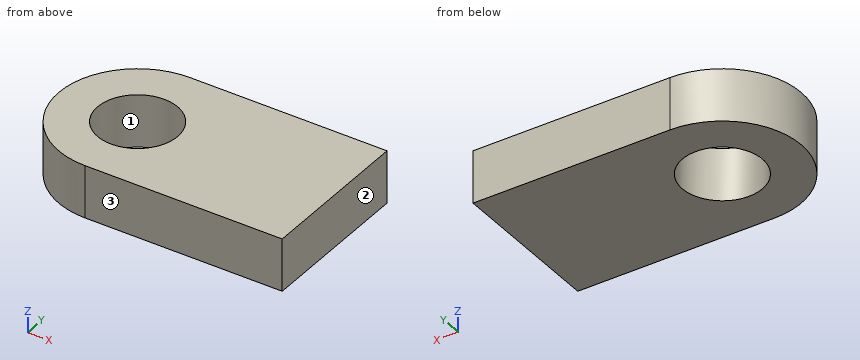
```python
from build123d import *

# Parameters (mm, degrees)
SKETCH_1_R      = 6.1
EXTRUDE_1_DEPTH = 4


with BuildPart() as part:
    # 草图1 → 凸台-拉伸1 (new, symmetric)
    with BuildSketch(Plane.XY):
        with BuildLine():
            Line((0, 12), (30, 12))
            Line((30, 12), (30, -12))
            Line((30, -12), (0, -12))
            ThreePointArc((0, -12), (-12, 0), (0, 12))
        make_face()
        Circle(SKETCH_1_R, mode=Mode.SUBTRACT)
    extrude(amount=EXTRUDE_1_DEPTH, both=True)


solid = part.part
```
Here's how the part is built. I have some questions about the finished solid (model axes, mm). Face numbers are marked on the shaded views. Give positions to 0.01 mm unless a question says otherwise; leave off trailing zeros. Write each loop counter-clockwise with the first axis right and the second up, starting at its lowest first coordinate (ties: lowest second). Pieces come first, ordered by that corner, then holes.
(1) Imagine slicing it at B-B, the plane z = -1.5. Write out the boundary of the cut face in (x, y).
Output values:
outline: (0, -12) - (30, -12) - (30, 12) - (0, 12) arc R12 ccw to start; hole circle Ø12.2 at (0, 0)
(2) If I drill on L1, parallel to Y at x = -1, z = -0.75; L2, parallel to X at y = 2.75, z = -2.25; L3, parallel to X at y = 1.75, z = -2.75, over which ranges is the centre line in solid material (lowest first)?
Output values:
L1: y = -11.96 to -6.02, 6.02 to 11.96
L2: x = -11.68 to -5.44, 5.44 to 30
L3: x = -11.87 to -5.84, 5.84 to 30
(3) Imagine slicing it at D-D, the plane y = -7.75. Write out the boundary of the cut face in (x, z), and give its area (3 significant figures).
Output values:
outline: (-9.16, -4) - (30, -4) - (30, 4) - (-9.16, 4) - close
area: 313 mm2
(4) Imagine slicing it at C-C, the plane x = -5. Write out the boundary of the cut face in (y, z), and give its area (3 significant figures).
Output values:
outline: (-10.91, -4) - (-3.49, -4) - (-3.49, 4) - (-10.91, 4) - close; (3.49, -4) - (10.91, -4) - (10.91, 4) - (3.49, 4) - close
area: 119 mm2
(5) Thinking about a two-plate mould opening in X: for the marked faces 1, 2 and 3, which applies, pulls with the +X half, pulls with the -X half, needs draft (parallel to the pull), parting line crosses it, or undercut?
Output values:
face 1: undercut
face 2: pulls with the +X half
face 3: needs draft
(6) Imagine slicing it at A-A, the plane y = 0. Write out the boundary of the cut face in (x, z).
Output values:
outline: (-12, -4) - (-6.1, -4) - (-6.1, 4) - (-12, 4) - close; (6.1, -4) - (30, -4) - (30, 4) - (6.1, 4) - close
